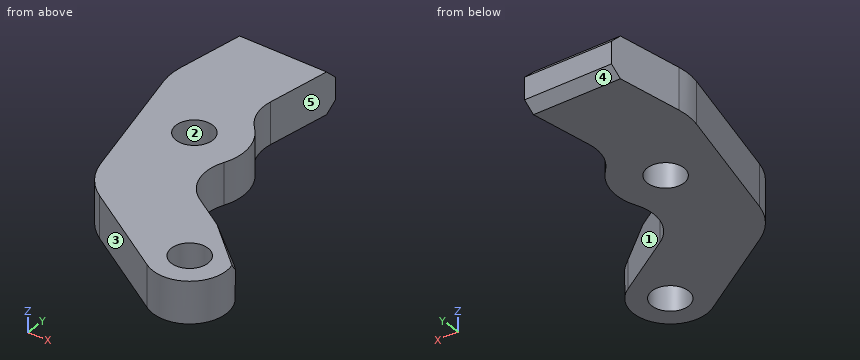
```python
from build123d import *

# Parameters (mm, degrees)
EXTRUDE_1_DEPTH                      = 34
CHAMFER_1_SIZE                       = 8
SKETCH_2_R                           = 15
CUT_EXTRUDE_1_DEPTH                  = 275.378242911
FILLET_2_R                           = 35
FILLET_4_R                           = 50
CUT_EXTRUDE_2_REACH                  = 275.869
CUT_EXTRUDE_2_DIRECTION_2_REACH      = 275.869
CUT_EXTRUDE_2_DIRECTION_2_END_RADIUS = 30


with BuildPart() as part:
    # 草图1 → 凸台-拉伸1 (new body)
    with BuildSketch(Plane.XY):
        with BuildLine():
            Line((-125, 235), (-53.92, 235))
            Line((-53.92, 235), (-68.018431876, 155.043819614))
            ThreePointArc((-68.018431876, 155.043819614), (-43.495979684, 123.54341), (-58.429747026, 86.521672326))
            ThreePointArc((-58.429747026, 86.521672326), (-63.94761811, 82.888703808), (-69.988207372, 80.21351355))
            Line((-69.988207372, 80.21351355), (16.130569268, 25.294361725))
            ThreePointArc((16.130569268, 25.294361725), (25.294361725, -16.130569268), (-16.130569268, -25.294361725))
            Line((-16.130569268, -25.294361725), (-106.728157023, 32.480990771))
            Line((-106.728157023, 32.480990771), (-137.486072687, 164.187962972))
            Line((-137.486072687, 164.187962972), (-125, 235))
        make_face()
    extrude(amount=EXTRUDE_1_DEPTH)

    # 倒角1
    chamfer_1_edges = [part.edges().sort_by_distance(p)[0] for p in [
        (-89.46, 235, 34),
        (-89.46, 235, 0),
    ]]
    chamfer(chamfer_1_edges, length=CHAMFER_1_SIZE)

    # 草图2 → 切除-拉伸1 (cut, through all)
    with BuildSketch(Plane(origin=(0, 0, 0), x_dir=(-1, 0, 0), z_dir=(0, 0, -1))):
        with Locations((0.008418778, 0)):
            Circle(SKETCH_2_R)
        with Locations((83.120594515, 118)):
            Circle(SKETCH_2_R)
    extrude(amount=-CUT_EXTRUDE_1_DEPTH, mode=Mode.SUBTRACT)

    # 圆角2
    fillet_2_edges = [part.edges().sort_by_distance(p)[0] for p in [
        (-69.988207372, 80.21351355, 17),
        (-68.018431876, 155.043819614, 17),
    ]]
    fillet(fillet_2_edges, radius=FILLET_2_R)

    # 圆角4
    fillet_4_edges = [part.edges().sort_by_distance(p)[0] for p in [
        (-106.728157023, 32.480990771, 17),
        (-137.486072687, 164.187962972, 17),
    ]]
    fillet(fillet_4_edges, radius=FILLET_4_R)

    # 切除-拉伸2: up to this plane
    cut_extrude_2_end = Plane(origin=(-69.988207372, 80.21351355, 34), z_dir=(-0.5376856422770575, -0.8431453908366625, 0))
    # 草图4 → 切除-拉伸2 (cut, up to the surface)
    with BuildSketch(Plane(origin=(0, 0, 0), x_dir=(0, 0, -1), z_dir=(0.7431448254773932, -0.6691306063588595, 0)), mode=Mode.PRIVATE) as cut_extrude_2_sk1:
        Polygon((-34, 25), (-22, 30), (-34, 30), align=None)
    cut_extrude_2_tool1 = split(extrude(cut_extrude_2_sk1.sketch, amount=-CUT_EXTRUDE_2_REACH, mode=Mode.PRIVATE), bisect_by=cut_extrude_2_end, keep=Keep.BOTH, mode=Mode.PRIVATE)
    add(cut_extrude_2_tool1.solids().sort_by_distance((18.958701, 21.05577, 30))[0], mode=Mode.SUBTRACT)

    # 切除-拉伸2 direction 2: up to this cylinder (the profile starts inside it)
    cut_extrude_2_direction_2_end = Plane(origin=(0, 0, 30), z_dir=(0, 0, -1)) * Cylinder(CUT_EXTRUDE_2_DIRECTION_2_END_RADIUS, 612.738, mode=Mode.PRIVATE)
    # 草图4 → 切除-拉伸2 direction 2 (cut, up to the surface)
    with BuildSketch(Plane(origin=(0, 0, 0), x_dir=(0, 0, -1), z_dir=(0.7431448254773932, -0.6691306063588595, 0)), mode=Mode.PRIVATE) as cut_extrude_2_direction_2_sk1:
        Polygon((-34, 25), (-22, 30), (-34, 30), align=None)
    cut_extrude_2_direction_2_tool1 = extrude(cut_extrude_2_direction_2_sk1.sketch, amount=CUT_EXTRUDE_2_DIRECTION_2_REACH, mode=Mode.PRIVATE) & cut_extrude_2_direction_2_end
    add(cut_extrude_2_direction_2_tool1.solids().sort_by_distance((18.958701, 21.05577, 30))[0], mode=Mode.SUBTRACT)


solid = part.part
```
Here's how the part is built. I have some questions about the finished solid (model axes, mm). Face numbers are marked on the shaded views. A direction names the side the tool comes from. Give positions to 0.01 mm unless a question says otherwise; leave off trailing zeros. Order: outer loops, then holes, each group sorted by start corner. A loop starts at its lowest first (then second) coordinate and runs counter-clockwise, first axis right, second up. Notation, with made-up numbers: (68.25, 39.25) - (96.25, 39.25) arc R20 cw to (96.25, 48.25) - close; hole circle Ø6 at (33.5, -23). An arc over 180 degrees is marked (long way). Answer as a JSON object with one key per item and string values. Group by question number.
Item 1: If we mould it in two halves opening along Y, with no side actions, what happens to the marked faces 1, 2 and 3? For each: pulls with the +Y half, pulls with the -Y half, needs draft (parallel to the pull), parting line crosses it, or undercut.
Item 2: If we section it at D-D on y = 0: Please give me the cut outline in (x, z), and give its area (3 significant figures).
Item 3: Which directions (+Z, -Z, +X, -X, +Y, -Y) give clear straight access to the entire face, cutting with the end or side of a thin tool? Please do the marked faces 4 and 5.
Item 4: Please list where these lines run through material, in increasing order: probe 1 along Y at (x, z) = (-5.5, 16); probe 2 along X at (y, z) = (-10.5, 29); probe 3 along X at (y, z) = (117.5, 2).
Item 5: If we section it at A-A on y = 118: Please give me the cut outline in (x, z), and give its area (3 significant figures).
Item 6: If we section it at C-C on x = 0: Please give me the cut outline in (y, z).
Item 7: If we section it at B-B on x = -82: Please give me the cut outline in (y, z), and give its area (3 significant figures).
Item 8: For P1, Ø4, axis at x = 3, z = 29.5, coming from the +Y side; P2, Ø12, axis at y = 49.5, z = 27.5, coming from the +X side; P3, Ø1, axis at y = 170.5, z = 5, coming from the +X side; P4, Ø5, axis at x = -43, y = 8.5, coming from the -Z side, each with a flat end and sliding along its axis, tell me the tip position at first contact or that it passes through.
Result set:
{
 "1": {"face 1": "pulls with the +Y half", "face 2": "undercut", "face 3": "pulls with the -Y half"},
 "2": {"outline": "(-55.79, 0) - (-15.01, 0) - (-15.01, 34) - (-55.79, 34) - close; (14.99, 0) - (30, 0) - (30, 34) - (14.99, 34) - close", "area": "1,900 mm²"},
 "3": {"face 4": "-Z, +X, -X, +Y", "face 5": "+Z, -Z, +X"},
 "4": {"probe 1": "-29.49 to -13.96, 13.96 to 39.09", "probe 2": "-39.33 to -10.72, 10.7 to 28.1", "probe 3": "-126.58 to -98.11, -68.13 to -43.11"},
 "5": {"outline": "(-126.7, 0) - (-98.12, 0) - (-98.12, 34) - (-126.7, 34) - close; (-68.12, 0) - (-43.11, 0) - (-43.11, 34) - (-68.12, 34) - close", "area": "1,820 mm²"},
 "6": {"outline": "(-30, 0) - (-15, 0) - (-15, 34) - (-30, 34) - close; (15, 0) - (35.58, 0) - (35.58, 30.54) - (33.64, 34) - (15, 34) - close"},
 "7": {"outline": "(16.71, 0) - (103.04, 0) - (103.04, 34) - (16.71, 34) - close; (132.96, 0) - (227, 0) - (235, 8) - (235, 26) - (227, 34) - (132.96, 34) - close", "area": "6,340 mm²"},
 "8": {"P1": "y = 34.94", "P2": "x = -12.42", "P3": "x = -64.72", "P4": "z = 0"}
}
